```python
from build123d import *

# Parameters (mm, degrees)
SKETCH1_R           = 1
BOSS_EXTRUDE1_DEPTH = 490
SKETCH2_R           = 3
BOSS_EXTRUDE2_DEPTH = 3
CHAMFER1_SIZE       = 0.2


with BuildPart() as part:
    # Sketch1 → Boss-Extrude1 (new body)
    with BuildSketch(Plane.XY):
        Circle(SKETCH1_R)
    extrude(amount=BOSS_EXTRUDE1_DEPTH)

    # Sketch2 → Boss-Extrude2 (add)
    with BuildSketch(Plane(origin=(0, 0, 0), x_dir=(-1, 0, 0), z_dir=(0, 0, -1))):
        Circle(SKETCH2_R)
    extrude(amount=BOSS_EXTRUDE2_DEPTH)

    # Chamfer1
    chamfer1_edges = [part.edges().sort_by_distance(p)[0] for p in [
        (3, 0, 0),
        (3, 0, -3),
    ]]
    chamfer(chamfer1_edges, length=CHAMFER1_SIZE)


solid = part.part
```
Verification items for the finished model (mm, model axes). Round coordinates to 2 decimals unless told otherwise and drop trailing zeros. Order: outer loops, then holes, each group sorted by start corner. A loop starts at its lowest first (then second) coordinate and runs counter-clockwise, first axis right, second up. Notation, with made-up numbers: (-6.75, 17) -> (31.25, 17) arc R19 cw to (31.25, 24) -> close; hole circle Ø6 at (-22, 34.25). An arc over 180 degrees is marked (long way). Put each result on its own line as item: value. Start each with the question number.
(1) Section check C-C (z = 250.5). Enter the section's corners in (x, y), then the cut area to 3 significant figures.
(2) Depth check by flat-ended pin: pin 1 Ø2 at (y, z) = (0.5, 278.5) entering from +X. Enter the tip coordinate at first touch or a pass-through.
(3) Material ranges on line 1 along Z through (x, y) = (-2.2, 0.75); line 2 along X through (y, z) = (-0.15, 230); line 3 along Z through (x, y) = (2.7, -1), recorded low to high.
(4) Section check A-A (y = 0). Enter the section's corners in (x, z), then the cut area to 3 significant figures.
Completed:
1. outline: circle Ø2 at (0, 0)
1. area: 3.14 mm2
2. pin 1: stops at x = 1
3. line 1: z = -3 to 0
3. line 2: x = -0.99 to 0.99
3. line 3: z = -2.92 to -0.08
4. outline: (-3, -2.8) -> (-2.8, -3) -> (2.8, -3) -> (3, -2.8) -> (3, -0.2) -> (2.8, 0) -> (1, 0) -> (1, 490) -> (-1, 490) -> (-1, 0) -> (-2.8, 0) -> (-3, -0.2) -> close
4. area: 998 mm2
